Geometry check sheet. Reference: the model listing, model coordinates, mm. Round coordinates to 2 decimals unless told otherwise and drop trailing zeros. Order: outer loops, then holes, each group sorted by start corner. A loop starts at its lowest first (then second) coordinate and runs counter-clockwise, first axis right, second up.
```python
from build123d import *

# Parameters (mm, degrees)
SKETCH1_W           = 30
SKETCH1_H           = 65
BOSS_EXTRUDE1_DEPTH = 800
CUT_EXTRUDE1_DEPTH  = 800


with BuildPart() as part:
    # Sketch1 → Boss-Extrude1 (new body)
    with BuildSketch(Plane.XY):
        with Locations((-25.852518101, 6.473439942)):
            Rectangle(SKETCH1_W, SKETCH1_H)
    extrude(amount=BOSS_EXTRUDE1_DEPTH)

    # Sketch2 → Cut-Extrude1 (cut)
    with BuildSketch(Plane.XY.offset(800)):
        Polygon((-37.852518101, 35.207148711), (-37.852518101, -23.026560058), (-13.852518101, -23.026560058), (-13.852518101, 35.973439942), (-37.852518101, 35.973439942), align=None)
    extrude(amount=-CUT_EXTRUDE1_DEPTH, mode=Mode.SUBTRACT)


solid = part.part
```
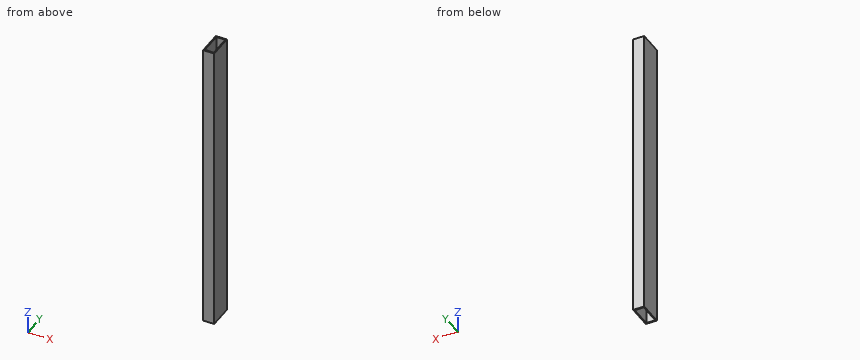
(1) Sectioned sample at C-C, the plane z = 553. Record the cut outline in (x, y), and give its area (3 significant figures).
Returned:
outline: (-40.85, -26.03) - (-10.85, -26.03) - (-10.85, 38.97) - (-40.85, 38.97) - close; hole (-37.85, -23.03) - (-13.85, -23.03) - (-13.85, 35.97) - (-37.85, 35.97) - close
area: 534 mm2
(2) Depth check by flat-ended pin: P1, Ø10, axis at x = -35, y = 3.5, coming from the -Z side; P2, Ø4, axis at x = -34.5, y = 31.5, coming from the +Z side. Enter the tip coordinate at first touch or a pass-through.
Returned:
P1: stops at z = 0
P2: passes through
(3) Sectioned sample at A-A, the plane x = -23.25. Record the cut outline in (y, z).
Returned:
outline: (-26.03, 0) - (-23.03, 0) - (-23.03, 800) - (-26.03, 800) - close; (35.97, 0) - (38.97, 0) - (38.97, 800) - (35.97, 800) - close
(4) Material ranges on line 1 (X direction, y = 33.5, z = 595); line 2 (Y direction, x = -35.5, z = 565.5), recorded low to high.
Returned:
line 1: x = -40.85 to -37.85, -13.85 to -10.85
line 2: y = -26.03 to -23.03, 35.97 to 38.97
(5) Sectioned sample at B-B, the plane y = 25. Record the cut outline in (x, z), and give its area (3 significant figures).
Returned:
outline: (-40.85, 0) - (-37.85, 0) - (-37.85, 800) - (-40.85, 800) - close; (-13.85, 0) - (-10.85, 0) - (-10.85, 800) - (-13.85, 800) - close
area: 4,800 mm2
